The listing builds one solid part. Answer for the finished solid, in the listing's coordinates (mm). Face numbers are marked on the shaded views. A direction names the side the tool comes from. Give positions to 0.01 mm unless a question says otherwise; leave off trailing zeros. Loops run counter-clockwise (first coordinate to the right, second up) from the corner with the lowest first, then second, coordinate; pieces in that order, holes last. Notation, with made-up numbers: M -27.75,39.5 L 27.25,39.5 A22 cw 27.25,63.5 Z; hole C -2.5,-5 d2. An arc over 180 degrees is marked long. Return JSON: item names as keys, results as strings.
from build123d import *

# Parameters (mm, degrees)
SKETCH1_R           = 10
BOSS_EXTRUDE1_DEPTH = 8
SKETCH2_R           = 8.5
CUT_EXTRUDE1_DEPTH  = 6
SKETCH3_R           = 3
CUT_EXTRUDE2_DEPTH  = 16.362291496
SKETCH4_R           = 9.25
CUT_EXTRUDE3_DEPTH  = 5


with BuildPart() as part:
    # Sketch1 → Boss-Extrude1 (new body)
    with BuildSketch(Plane.XY):
        Circle(SKETCH1_R)
    extrude(amount=BOSS_EXTRUDE1_DEPTH)

    # Sketch2 → Cut-Extrude1 (cut)
    with BuildSketch(Plane.XY.offset(8)):
        Circle(SKETCH2_R)
    extrude(amount=-CUT_EXTRUDE1_DEPTH, mode=Mode.SUBTRACT)

    # Sketch3 → Cut-Extrude2 (cut, through all)
    with BuildSketch(Plane.XY.offset(2)):
        Circle(SKETCH3_R)
    extrude(amount=-CUT_EXTRUDE2_DEPTH, mode=Mode.SUBTRACT)

    # Sketch4 → Cut-Extrude3 (cut)
    with BuildSketch(Plane.XY.offset(2)):
        Circle(SKETCH4_R)
    extrude(amount=CUT_EXTRUDE3_DEPTH, mode=Mode.SUBTRACT)


solid = part.part
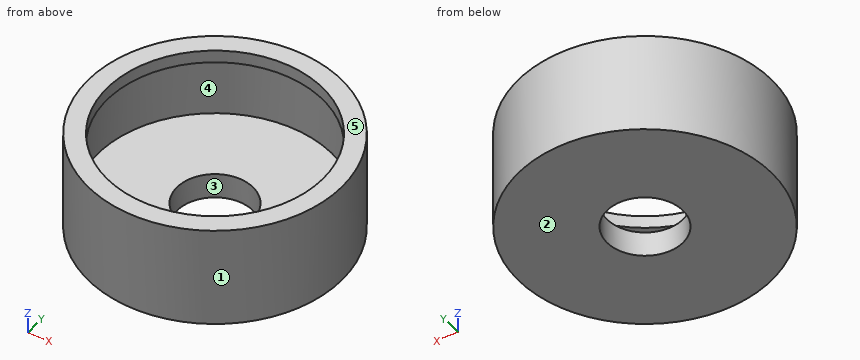
(1) The part is cut by section D-D (x = -5.75). Determine the outline of the cut face in (y, z).
Values follow:
{"outline": "M -8.18,0 L 8.18,0 L 8.18,8 L 6.26,8 L 6.26,7 L 7.25,7 L 7.25,2 L -7.25,2 L -7.25,7 L -6.26,7 L -6.26,8 L -8.18,8 Z"}
(2) Straight lines are drawn through the part: line 1 along Y through (x, z) = (0, 7.35); line 2 along Y through (x, z) = (0, 5.5); line 3 along Z through (x, y) = (3.5, 0.5). For each, find the intervals that lie inside material, in ascending order.
Values follow:
{"line 1": "-10 to -8.5, 8.5 to 10", "line 2": "-10 to -9.25, 9.25 to 10", "line 3": "0 to 2"}
(3) A tool of negligible diameter and unlimited length cuts with its end or side. For the marked faces 4 and 5, from which of +Z, -Z, +X, -X, +Y, -Y can it reach the whole face along a straight path? Write none if from no direction.
Values follow:
{"face 4": "none", "face 5": "+Z, +X, -X, +Y, -Y"}
(4) Determine the mould class of the marked faces 1, 2 and 3 for opening direction X: released by +X, released by -X, zero draft, split by the parting line, or undercut.
Values follow:
{"face 1": "split by the parting line", "face 2": "zero draft", "face 3": "undercut"}
(5) Given pin 1 (1 mm diameter, centred on y = -3.5, z = 4, fed in from -X); pin 2 (2 mm diameter, centred on y = -5.5, z = 3.5, fed in from +X); pin 3 (4 mm diameter, centred on x = 6.5, z = 2.5, fed in from +Y), each flat-ended and moving along its own axis, determine where each tip first touches the part or whether it passes through.
Values follow:
{"pin 1": "x = -9.54", "pin 2": "x = 8.93", "pin 3": "y = 8.93"}
(6) The part is cut by section C-C (z = 5.75). Determine the outline of the cut face in (x, y).
Values follow:
{"outline": "C 0,0 d20; hole C 0,0 d18.5"}
(7) The part is cut by section A-A (y = 0). Determine the outline of the cut face in (x, z).
Values follow:
{"outline": "M -10,0 L -3,0 L -3,2 L -9.25,2 L -9.25,7 L -8.5,7 L -8.5,8 L -10,8 Z; M 3,0 L 10,0 L 10,8 L 8.5,8 L 8.5,7 L 9.25,7 L 9.25,2 L 3,2 Z"}
